```python
from build123d import *

# Parameters (mm, degrees)
SKETCH4_R           = 12.25
BOSS_EXTRUDE1_DEPTH = 51
SKETCH5_W           = 5
SKETCH5_H           = 2.5
SKETCH5_R           = 0.9
BOSS_EXTRUDE2_DEPTH = 0.5
FILLET1_R           = 1
SKETCH6_R           = 3
BOSS_EXTRUDE3_DEPTH = 2.5
SKETCH7_R           = 2
BOSS_EXTRUDE4_DEPTH = 12
SKETCH8_W           = 2
SKETCH8_H           = 3.5
SKETCH9_R           = 1.6
CUT_EXTRUDE1_DEPTH  = 5


with BuildPart() as part:
    # Sketch4 → Boss-Extrude1 (new body)
    with BuildSketch(Plane(origin=(0, 0, 0), x_dir=(0, 0, -1), z_dir=(1, 0, 0))):
        Circle(SKETCH4_R)
    extrude(amount=BOSS_EXTRUDE1_DEPTH)

    # Sketch5 → Boss-Extrude2 (add, symmetric)
    # profile 1 of 2: a face of its own
    with BuildSketch(Plane.XY):
        with Locations((-2.5, 9.653593257)):
            Rectangle(SKETCH5_W, SKETCH5_H)
        with Locations((-2.5, 9.653593257)):
            Circle(SKETCH5_R, mode=Mode.SUBTRACT)
    # profile 2 of 2: a face of its own
    with BuildSketch(Plane.XY):
        with Locations((-2.5, -9.653593257)):
            Rectangle(SKETCH5_W, SKETCH5_H)
        with Locations(Location((-2.5, -9.653593257, 0), (0, 0, 180))):
            Circle(SKETCH5_R, mode=Mode.SUBTRACT)
    extrude(amount=BOSS_EXTRUDE2_DEPTH, both=True)

    # Fillet1
    fillet1_edges = [part.edges().sort_by_distance(p)[0] for p in [
        (-5, 8.403593257, 0),
        (-5, -8.403593257, 0),
        (-5, -10.903593257, 0),
        (-5, 10.903593257, 0),
    ]]
    fillet(fillet1_edges, radius=FILLET1_R)

    # Sketch6 → Boss-Extrude3 (add)
    with BuildSketch(Plane(origin=(51, 0, 0), x_dir=(0, 0, -1), z_dir=(1, 0, 0))):
        Circle(SKETCH6_R)
    extrude(amount=BOSS_EXTRUDE3_DEPTH)

    # Sketch7 → Boss-Extrude4 (add)
    with BuildSketch(Plane(origin=(53.5, 0, 0), x_dir=(0, 0, -1), z_dir=(1, 0, 0))):
        Circle(SKETCH7_R)
    extrude(amount=BOSS_EXTRUDE4_DEPTH)

    # Sketch8 → Cut-Revolve1 (revolve, cut)
    with BuildSketch(Plane.XY, mode=Mode.PRIVATE) as cut_revolve1_sk:
        with Locations((14.235706655, 13.25)):
            Rectangle(SKETCH8_W, SKETCH8_H)
    revolve(cut_revolve1_sk.sketch.rotate(Axis((-4.366287434, 0, 0), (1, 0, 0)), 90), axis=Axis((-4.366287434, 0, 0), (1, 0, 0)), mode=Mode.SUBTRACT)

    # Sketch9 → Cut-Extrude1 (cut)
    with BuildSketch(Plane(origin=(51, 0, 0), x_dir=(0, 0, -1), z_dir=(1, 0, 0))):
        with Locations((-8.5, 0)):
            Circle(SKETCH9_R)
        with Locations((8.5, 0)):
            Circle(SKETCH9_R)
    extrude(amount=-CUT_EXTRUDE1_DEPTH, mode=Mode.SUBTRACT)


solid = part.part
```
CAD build for the part. Positions are in the model's coordinates, mm. A direction names the side the tool comes from. Coordinates: 2 decimals unless noted, no trailing zeros. Write each loop counter-clockwise with the first axis right and the second up, starting at its lowest first coordinate (ties: lowest second). Pieces come first, ordered by that corner, then holes. Notation, with made-up numbers: (54, 58.5) -> (91, 58.5) arc R16 ccw to (91, 78.5) -> close; hole circle Ø9 at (51, -27). An arc over 180 degrees is marked (long way). Use CSV: the item, a comma, the result in double quotes. Start each with the question number.
Item 1: Two-plate mould, pull along X, no slides. Class faces 1 (the flat face through (15.236, -11, -4)), 2 (the flat face through (0, 0, 0)), 3 (the cylindrical face through (32.868, 10.329, -6.586)), 4 (the cylindrical face through (-2.617, 10.546, -0.007)): +X half, -X half, draft (parallel to the pull), parting line (faces both ways), or undercut.
Item 2: Band-saw the part on A-A, the plane x = -2.5. Write the cut outline in (y, z), plus the area to 3 significant figures.
Item 3: Tool access for faces 5 (the flat face through (51, -3, -3)), 6 (the flat face through (-1, -10, 0.5)), 7 (the cylindrical face through (14.2, -11.4, -1.5)), 8 (the flat face through (-1, -10, -0.5)): list every direction of +Z, -Z, +X, -X, +Y, -Y with a clear straight run to the whole face (end or side of a thin tool).
Item 4: Band-saw the part on D-D, the plane x = 31.5. Write the cut outline in (y, z).
Item 5: Band-saw the part on C-C, the plane z = 9.25. Write the cut outline in (x, y).
Item 6: Band-saw the part on B-B, the plane y = 0. Write the cut outline in (x, z).
Item 7: Wall check: probe 1 along Y at (x, z) = (-2.5, 0.1); probe 2 along X at (y, z) = (-9.5, 7); probe 3 along X at (y, z) = (2.5, 4.25). Give the ranges that are in metal, low to high.
Item 8: Drop flat-ended pins along their axis: P1, Ø1.2, axis at x = -3.5, y = 10, coming from the +Z side; P2, Ø1, axis at y = 0, z = 9, coming from the +X side; P3, Ø1.2, axis at x = -2, y = -10, coming from the -Z side. Give the stop position or say it passes through.
Response values:
1,face 1,"undercut"
1,face 2,"-X half"
1,face 3,"draft"
1,face 4,"undercut"
2,outline,"(-10.9, -0.5) -> (-10.55, -0.5) -> (-10.55, 0.5) -> (-10.9, 0.5) -> close; (-8.75, -0.5) -> (-8.4, -0.5) -> (-8.4, 0.5) -> (-8.75, 0.5) -> close; (8.4, -0.5) -> (8.75, -0.5) -> (8.75, 0.5) -> (8.4, 0.5) -> close; (10.55, -0.5) -> (10.9, -0.5) -> (10.9, 0.5) -> (10.55, 0.5) -> close"
2,area,"1.40 mm2"
3,face 5,"+X"
3,face 6,"+Z, -X, +Y, -Y"
3,face 7,"none"
3,face 8,"-Z, -X, +Y, -Y"
4,outline,"circle Ø24.5 at (0, 0)"
5,outline,"(0, -8.03) -> (13.24, -8.03) -> (13.24, -6.83) -> (15.24, -6.83) -> (15.24, -8.03) -> (51, -8.03) -> (51, -1.41) -> (46, -1.41) -> (46, 1.41) -> (51, 1.41) -> (51, 8.03) -> (15.24, 8.03) -> (15.24, 6.83) -> (13.24, 6.83) -> (13.24, 8.03) -> (0, 8.03) -> close"
6,outline,"(0, -12.25) -> (13.24, -12.25) -> (13.24, -11.5) -> (15.24, -11.5) -> (15.24, -12.25) -> (51, -12.25) -> (51, -10.1) -> (46, -10.1) -> (46, -6.9) -> (51, -6.9) -> (51, -3) -> (53.5, -3) -> (53.5, -2) -> (65.5, -2) -> (65.5, 2) -> (53.5, 2) -> (53.5, 3) -> (51, 3) -> (51, 6.9) -> (46, 6.9) -> (46, 10.1) -> (51, 10.1) -> (51, 12.25) -> (15.24, 12.25) -> (15.24, 11.5) -> (13.24, 11.5) -> (13.24, 12.25) -> (0, 12.25) -> close"
7,probe 1,"y = -10.9 to -10.55, -8.75 to -8.4, 8.4 to 8.75, 10.55 to 10.9"
7,probe 2,"x = 0 to 13.24, 15.24 to 51"
7,probe 3,"x = 0 to 51"
8,P1,"stops at z = 0.5"
8,P2,"stops at x = 46"
8,P3,"stops at z = -0.5"
